Design review of the part built by this model. Coordinates are the model's own, in mm. Coordinates: 2 decimals unless noted, no trailing zeros. Loops run counter-clockwise (first coordinate to the right, second up) from the corner with the lowest first, then second, coordinate; pieces in that order, holes last. Notation, with made-up numbers: (84, 15.5) -> (101, 15.5) arc R21 ccw to (101, 31.5) -> close; hole circle Ø3 at (55, -38). An arc over 180 degrees is marked (long way). Answer in a Markdown table with one row per item.
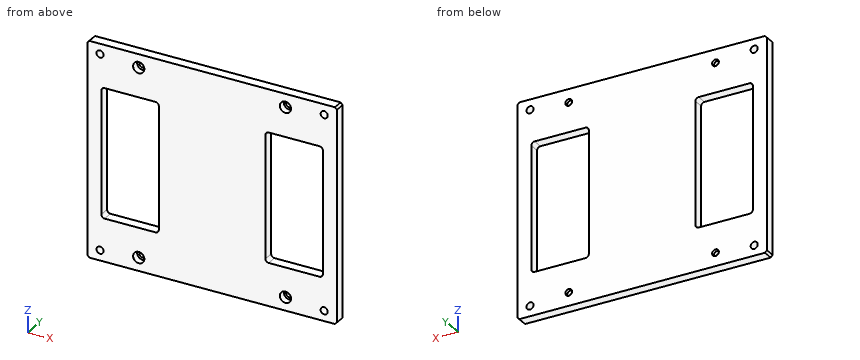
```python
from build123d import *

# Parameters (mm, degrees)
SKETCH_1_W          = 245
SKETCH_1_H          = 210
EXTRUDE_1_DEPTH     = 10
CHAMFER_1_SIZE      = 2
CUT_EXTRUDE_1_REACH = 163.652
SKETCH_5_R          = 3.5
CUT_EXTRUDE_2_REACH = 163.652


with BuildPart() as part:
    # 草图1 → 凸台-拉伸1 (new body)
    with BuildSketch(Plane(origin=(0, 0, 0), x_dir=(1, 0, 0), z_dir=(0, 1, 0))):
        Rectangle(SKETCH_1_W, SKETCH_1_H)
    extrude(amount=EXTRUDE_1_DEPTH)

    # 倒角1
    chamfer_1_edges = [part.edges().sort_by_distance(p)[0] for p in [
        (122.5, 5, 105),
        (-122.5, 5, 105),
        (-122.5, 5, -105),
        (122.5, 5, -105),
    ]]
    chamfer(chamfer_1_edges, length=CHAMFER_1_SIZE)

    # 草图4 → 打孔尺寸(%根据)内六角圆柱头螺钉的类型1 (revolve, cut)
    with BuildSketch(Plane(origin=(72, 0, 92), x_dir=(0, 0, -1), z_dir=(1, 0, 0))):
        Polygon((0, 0), (0, 10.001), (3.3, 10.001), (3.3, 6.8), (5.5, 6.8), (5.5, 0.025), (5.525, 0), align=None)
    hole_wizard_1 = revolve(axis=Axis((72, -6.35, 92), (0, 1, 0)), mode=Mode.SUBTRACT)

    # 镜向1: 打孔尺寸(%根据)内六角圆柱头螺钉的类型1 across plane
    add(hole_wizard_1.mirror(Plane(origin=(0, 0, 0), x_dir=(0, 0, 1), z_dir=(1, 0, 0))), mode=Mode.SUBTRACT)

    # 镜向2: 打孔尺寸(%根据)内六角圆柱头螺钉的类型1 across plane
    add(hole_wizard_1.mirror(Plane.XY), mode=Mode.SUBTRACT)

    # 镜向2 copy 1 sketch → 镜向2 copy 1 (revolve, cut)
    with BuildSketch(Plane(origin=(-72, 0, -92), x_dir=(0, 0, 1), z_dir=(-1, 0, 0))):
        Polygon((0, 0), (0, 10.001), (3.3, 10.001), (3.3, 6.8), (5.5, 6.8), (5.5, 0.025), (5.525, 0), align=None)
    revolve(axis=Axis((-72, -6.35, -92), (0, 1, 0)), mode=Mode.SUBTRACT)

    # 草图5 → 切除-拉伸1 (cut, up to next)
    with BuildSketch(Plane(origin=(0, 10, 0), x_dir=(1, 0, 0), z_dir=(0, 1, 0)), mode=Mode.PRIVATE) as cut_extrude_1_sk1:
        with Locations(Location((-110, 95, 0), (0, 0, 270))):
            Circle(SKETCH_5_R)
    cut_extrude_1_tool1 = extrude(cut_extrude_1_sk1.sketch, amount=-CUT_EXTRUDE_1_REACH, mode=Mode.PRIVATE) & part.part
    # 草图5 → 切除-拉伸1 (cut, up to next)
    with BuildSketch(Plane(origin=(0, 10, 0), x_dir=(1, 0, 0), z_dir=(0, 1, 0)), mode=Mode.PRIVATE) as cut_extrude_1_sk2:
        with Locations(Location((110, 95, 0), (0, 0, 270))):
            Circle(SKETCH_5_R)
    cut_extrude_1_tool2 = extrude(cut_extrude_1_sk2.sketch, amount=-CUT_EXTRUDE_1_REACH, mode=Mode.PRIVATE) & part.part
    # 草图5 → 切除-拉伸1 (cut, up to next)
    with BuildSketch(Plane(origin=(0, 10, 0), x_dir=(1, 0, 0), z_dir=(0, 1, 0)), mode=Mode.PRIVATE) as cut_extrude_1_sk3:
        with Locations(Location((110, -95, 0), (0, 0, 270))):
            Circle(SKETCH_5_R)
    cut_extrude_1_tool3 = extrude(cut_extrude_1_sk3.sketch, amount=-CUT_EXTRUDE_1_REACH, mode=Mode.PRIVATE) & part.part
    # 草图5 → 切除-拉伸1 (cut, up to next)
    with BuildSketch(Plane(origin=(0, 10, 0), x_dir=(1, 0, 0), z_dir=(0, 1, 0)), mode=Mode.PRIVATE) as cut_extrude_1_sk4:
        with Locations(Location((-110, -95, 0), (0, 0, 270))):
            Circle(SKETCH_5_R)
    cut_extrude_1_tool4 = extrude(cut_extrude_1_sk4.sketch, amount=-CUT_EXTRUDE_1_REACH, mode=Mode.PRIVATE) & part.part
    add(cut_extrude_1_tool1.solids().sort_by_distance((-110, 10, -95))[0], mode=Mode.SUBTRACT)
    add(cut_extrude_1_tool2.solids().sort_by_distance((110, 10, -95))[0], mode=Mode.SUBTRACT)
    add(cut_extrude_1_tool3.solids().sort_by_distance((110, 10, 95))[0], mode=Mode.SUBTRACT)
    add(cut_extrude_1_tool4.solids().sort_by_distance((-110, 10, 95))[0], mode=Mode.SUBTRACT)

    # 草图6 → 切除-拉伸2 (cut, up to next)
    with BuildSketch(Plane(origin=(0, 10, 0), x_dir=(1, 0, 0), z_dir=(0, 1, 0)), mode=Mode.PRIVATE) as cut_extrude_2_sk1:
        with BuildLine():
            Line((105.5, -63.2), (55.5, -63.2))
            ThreePointArc((55.5, -63.2), (53.2372583, -62.2627417), (52.3, -60))
            Line((52.3, -60), (52.3, 60))
            ThreePointArc((52.3, 60), (53.2372583, 62.2627417), (55.5, 63.2))
            Line((55.5, 63.2), (105.5, 63.2))
            ThreePointArc((105.5, 63.2), (107.7627417, 62.2627417), (108.7, 60))
            Line((108.7, 60), (108.7, -60))
            ThreePointArc((108.7, -60), (107.7627417, -62.2627417), (105.5, -63.2))
        make_face()
    cut_extrude_2_tool1 = extrude(cut_extrude_2_sk1.sketch, amount=-CUT_EXTRUDE_2_REACH, mode=Mode.PRIVATE) & part.part
    cut_extrude_2 = cut_extrude_2_tool1.solids().sort_by_distance((80.5, 10, 0))[0]
    add(cut_extrude_2, mode=Mode.SUBTRACT)

    # 镜向3: 切除-拉伸2 across plane
    add(cut_extrude_2.mirror(Plane(origin=(0, 0, 0), x_dir=(0, 0, 1), z_dir=(1, 0, 0))), mode=Mode.SUBTRACT)


solid = part.part
```
(1) Take a section at C-C on y = 3. Count the separate pieces of the cut face and the enclosed holes in it, and give its area (3 significant figures).
Evaluation:
| item | result |
|---|---|
| separate pieces | 1 |
| enclosed holes | 10 |
| area | 36,700 mm² |
(2) To check wall thickness, follow probe 1 along X at (y, z) = (2.25, 19); probe 2 along Z at (x, y) = (86, 5.75); probe 3 along X at (y, z) = (1.5, -90.5). State the ranges of each line that lie inside material, in increasing order.
Evaluation:
| item | result |
|---|---|
| probe 1 | x = -122.5 to -108.7, -52.3 to 52.3, 108.7 to 122.5 |
| probe 2 | z = -105 to -63.2, 63.2 to 105 |
| probe 3 | x = -122.5 to -77.29, -66.71 to 66.71, 77.29 to 122.5 |
(3) Take a section at A-A on x = 72. Give the boundary of the cut face in (y, z) (3 decimals).
Evaluation:
| item | result |
|---|---|
| outline | (0, -105) -> (10, -105) -> (10, -95.3) -> (6.8, -95.3) -> (6.8, -97.5) -> (0.025, -97.5) -> (0, -97.525) -> close; (0, -86.475) -> (0.025, -86.5) -> (6.8, -86.5) -> (6.8, -88.7) -> (10, -88.7) -> (10, -63.2) -> (0, -63.2) -> close; (0, 63.2) -> (10, 63.2) -> (10, 88.7) -> (6.8, 88.7) -> (6.8, 86.5) -> (0.025, 86.5) -> (0, 86.475) -> close; (0, 97.525) -> (0.025, 97.5) -> (6.8, 97.5) -> (6.8, 95.3) -> (10, 95.3) -> (10, 105) -> (0, 105) -> close |
(4) Take a section at B-B on z = 33. Give the boundary of the cut face in (x, y).
Evaluation:
| item | result |
|---|---|
| outline | (-122.5, 0) -> (-108.7, 0) -> (-108.7, 10) -> (-122.5, 10) -> close; (-52.3, 0) -> (52.3, 0) -> (52.3, 10) -> (-52.3, 10) -> close; (108.7, 0) -> (122.5, 0) -> (122.5, 10) -> (108.7, 10) -> close |
(5) For pin 1 (5.5 mm diameter, centred on x = -69.5, z = -93, fed in from -Y); pin 2 (6.5 mm diameter, centred on x = 110, z = -95, fed in from -Y), all flat-tipped, find the tip position at first contact; note any pin that passes through.
Evaluation:
| item | result |
|---|---|
| pin 1 | stops at y = 6.8 |
| pin 2 | passes through |
